Verification items for the finished model (mm, model axes). A direction names the side the tool comes from. Coordinates: 2 decimals unless noted, no trailing zeros. Write each loop counter-clockwise with the first axis right and the second up, starting at its lowest first coordinate (ties: lowest second). Pieces come first, ordered by that corner, then holes. Notation, with made-up numbers: (-4.5, 80.25) - (11.5, 80.25) arc R13 ccw to (11.5, 96.25) - close; hole circle Ø1 at (48.5, 47). An arc over 180 degrees is marked (long way). Use one line per item in the form item = value. Start each with the question number.
(1) Material ranges on line 1 (Y direction, x = 0, z = 9); line 2 (Y direction, x = 0, z = 26); line 3 (X direction, y = -13.5, z = 4), recorded low to high. Write a range as [from, to].
(2) Sectioned sample at A-A (y = 0). Record the cut outline in (x, z).
(3) Sectioned sample at C-C (z = 14). Record the cut outline in (x, y).
(4) Gauge pin test, flat ends, axial feed: pin 1 Ø5 at (x, y) = (-29, -27) entering from -Z; pin 2 Ø12 at (y, z) = (26, 13) entering from +X; pin 3 Ø2 at (x, z) = (-4, 17) entering from -Y; pin 4 Ø6 at (x, z) = (25, 17.5) entering from -Y. Record the tip position at first contact, or that the pin passes through.
(5) Tool access check on faces 1 (the conical face through (-13.9, 26.73, 1.87)), 2 (the cylindrical face through (39.96, -1.76, 22.17)). Record the directions out of +Z, -Z, +X, -X, +Y, -Y that give a thin tool (end or side, any length) a straight path to the whole face; none if there is none.
(6) Mould release check, pull along X, two halves, no side actions. Record for faces 3 (the cylindrical face through (-37.874, 15.703, 5.944)), 4 (the cylindrical face through (-16.128, -25.296, 17.776)), 5 (the flat face through (6, -32, 0)): released by +X, released by -X, zero draft, split by the parting line, or undercut.
from build123d import *

# Parameters (mm, degrees)
SKETCH1_W     = 26
SKETCH1_H     = 10
SKETCH1_W_2   = 10
SKETCH1_H_2   = 1
CHAMFER1_SIZE = 2


with BuildPart() as part:
    # Sketch1 → Revolve1 (revolve)
    with BuildSketch(Plane(origin=(0, 0, 0), x_dir=(0, 0, -1), z_dir=(1, 0, 0)), mode=Mode.PRIVATE) as revolve1_sk:
        with Locations((-23, 35)):
            Rectangle(SKETCH1_W, SKETCH1_H)
        with Locations((-5, 35)):
            Rectangle(SKETCH1_W_2, SKETCH1_H)
        with Locations((-5, 40.5)):
            Rectangle(SKETCH1_W_2, SKETCH1_H_2)
    revolve(revolve1_sk.sketch.rotate(Axis((0, 0, 0), (0, 0, 1)), 90), axis=Axis((0, 0, 0), (0, 0, 1)))

    # Chamfer1
    chamfer1_edges = [part.edges().sort_by_distance(p)[0] for p in [
        (30, 0, 36),
        (40, 0, 36),
        (41, 0, 0),
        (30, 0, 0),
    ]]
    chamfer(chamfer1_edges, length=CHAMFER1_SIZE)


solid = part.part
Answers below:
q1.line_1 = [-41, -30], [30, 41]
q1.line_2 = [-40, -30], [30, 40]
q1.line_3 = [-38.71, -26.79], [26.79, 38.71]
q2.outline = (-41, 2) - (-39, 0) - (-32, 0) - (-30, 2) - (-30, 34) - (-32, 36) - (-38, 36) - (-40, 34) - (-40, 10) - (-41, 10) - close; (30, 2) - (32, 0) - (39, 0) - (41, 2) - (41, 10) - (40, 10) - (40, 34) - (38, 36) - (32, 36) - (30, 34) - close
q3.outline = circle Ø80 at (0, 0); hole circle Ø60 at (0, 0)
q4.pin_1 = 0
q4.pin_2 = 35.33
q4.pin_3 = -39.89
q4.pin_4 = -33.41
q5.face_1 = -Z
q5.face_2 = +Z
q6.face_3 = split by the parting line
q6.face_4 = undercut
q6.face_5 = zero draft
